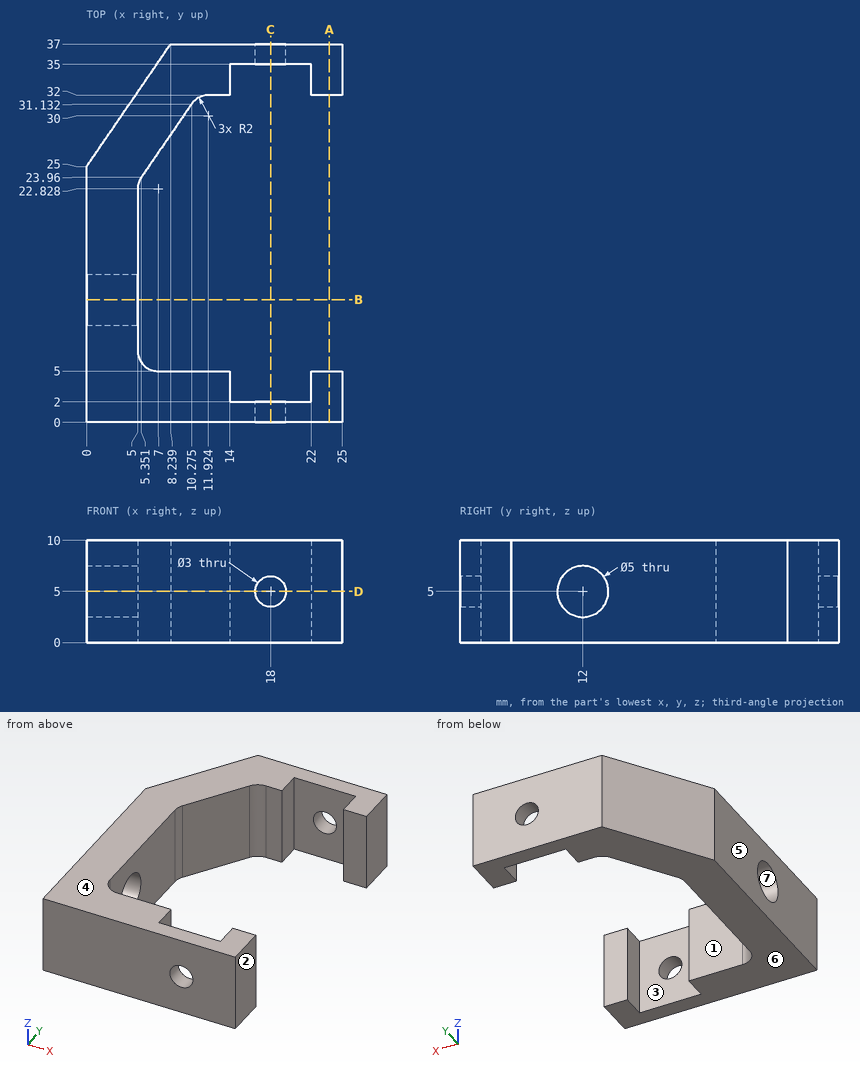
Input: dimensioned drawing with shaded views. Units: mm. Origin: part minimum x, y, z. A direction names the side the tool comes from. Coordinates: 2 decimals unless noted, no trailing zeros. Order: outer loops, then holes, each group sorted by start corner. A loop starts at its lowest first (then second) coordinate and runs counter-clockwise, first axis right, second up.
(1) First-contact query: pin 1 (1 mm diameter, centred on y = 28.5, z = 5, fed in from -X); pin 2 (6 mm diameter, centred on y = 13.5, z = 6, fed in from +X); pin 3 (2.5 mm diameter, centred on y = 33.5, z = 6, fed in from -X). Flat tips, straight axial feed; report the tip coordinate or a pass-through.
(2) Access query for the marked faces 1, 2 and 3. Directions: +Z, -Z, +X, -X, +Y, -Y. A direction counts if a zero-diameter tool reaches every point of the face in a straight line with its end or side. Return the directions, or none.
(3) Material intervals for probe 1 along Y at (x, z) = (23.75, 7.5); probe 2 along Y at (x, z) = (14.5, 4.25); probe 3 along X at (y, z) = (4.5, 2.25), sorted ascending.
(4) Section query D-D (z = 5). State how many separate pieces and enclosed holes the cut face has, plus the area to 3 significant figures.
(5) Section query C-C (x = 18). Return the cut outline in (y, z).
(6) Section query B-B (y = 12). Return the cut outline in (x, z), plus the area to 3 significant figures.
(7) Section query A-A (x = 23.75). Return the cut outline in (y, z), plus the area to 3 significant figures.
(8) Draft query along Z for the marked faces 4, 5, 6 and 7. Return one class per face: pulls with the +Z half, pulls with the -Z half, needs draft (parallel to the pull), parting line crosses it, or undercut.
Solution:
1. pin 1: stops at x = 2.06
1. pin 2: stops at x = 5
1. pin 3: stops at x = 4.98
2. face 1: +Z, -Z, +X
2. face 2: +Z, -Z, +X, +Y, -Y
2. face 3: +Z, -Z
3. probe 1: y = 0 to 5, 32 to 37
3. probe 2: y = 0 to 2, 35 to 37
3. probe 3: x = 0 to 14, 22 to 25
4. separate pieces: 4
4. enclosed holes: 0
4. area: 277 mm2
5. outline: (0, 0) - (2, 0) - (2, 3.5) - (0, 3.5) - close; (0, 6.5) - (2, 6.5) - (2, 10) - (0, 10) - close; (35, 0) - (37, 0) - (37, 3.5) - (35, 3.5) - close; (35, 6.5) - (37, 6.5) - (37, 10) - (35, 10) - close
6. outline: (0, 0) - (5, 0) - (5, 2.5) - (0, 2.5) - close; (0, 7.5) - (5, 7.5) - (5, 10) - (0, 10) - close
6. area: 25.0 mm2
7. outline: (0, 0) - (5, 0) - (5, 10) - (0, 10) - close; (32, 0) - (37, 0) - (37, 10) - (32, 10) - close
7. area: 100 mm2
8. face 4: pulls with the +Z half
8. face 5: needs draft
8. face 6: pulls with the -Z half
8. face 7: undercut
